```python
from build123d import *

# Parameters (mm, degrees)
HUB_BLOCK_SKETCH_R   = 32.5
HUB_BLOCK_SKETCH_R_2 = 26
HUB_BLOCK_DEPTH      = 35
ARM_PROFILE_SKETCH_R = 6.5
ARM_BODY_DEPTH       = 42


with BuildPart() as part:
    # Hub Block Sketch → Hub Block (new, symmetric)
    with BuildSketch(Plane.XY):
        Circle(HUB_BLOCK_SKETCH_R)
        Circle(HUB_BLOCK_SKETCH_R_2, mode=Mode.SUBTRACT)
    extrude(amount=HUB_BLOCK_DEPTH, both=True)

    # Arm Profile Sketch → Arm Body (add)
    with BuildSketch(Plane(origin=(0, 0, -21), x_dir=(-1, 0, 0), z_dir=(0, 0, -1))):
        with BuildLine():
            ThreePointArc((89.262059242, -14), (51.834907578, -24.492209287), (25.315908922, -52.910880046))
            ThreePointArc((25.315908922, -52.910880046), (16.763184773, -57.879874978), (7.189691393, -55.392260556))
            ThreePointArc((7.189691393, -55.392260556), (-14.44681941, -44.272249892), (-38.551485077, -40.992260556))
            ThreePointArc((-38.551485077, -40.992260556), (-49.467382276, -35.70933903), (-51.274422727, -23.717647059))
            ThreePointArc((-51.274422727, -23.717647059), (-47.255840909, 0), (-51.274422727, 23.717647059))
            ThreePointArc((-51.274422727, 23.717647059), (-49.467382276, 35.70933903), (-38.551485077, 40.992260556))
            ThreePointArc((-38.551485077, 40.992260556), (-14.44681941, 44.272249892), (7.189691393, 55.392260556))
            ThreePointArc((7.189691393, 55.392260556), (16.763184773, 57.879874978), (25.315908922, 52.910880046))
            ThreePointArc((25.315908922, 52.910880046), (51.834907578, 24.492209287), (89.262059242, 14))
            Line((89.262059242, 14), (239.5, 14))
            ThreePointArc((239.5, 14), (232.5, 0), (239.5, -14))
            Line((239.5, -14), (89.262059242, -14))
        make_face()
        with Locations((15, -45)):
            Circle(ARM_PROFILE_SKETCH_R, mode=Mode.SUBTRACT)
        with Locations((15, 45)):
            Circle(ARM_PROFILE_SKETCH_R, mode=Mode.SUBTRACT)
        with Locations((-39, -28)):
            Circle(ARM_PROFILE_SKETCH_R, mode=Mode.SUBTRACT)
        with Locations((-39, 28)):
            Circle(ARM_PROFILE_SKETCH_R, mode=Mode.SUBTRACT)
        with BuildLine():
            ThreePointArc((220, -7), (227, 0), (220, 7))
            Line((220, 7), (70, 7))
            ThreePointArc((70, 7), (63, 0), (70, -7))
            Line((70, -7), (220, -7))
        make_face(mode=Mode.SUBTRACT)
    extrude(amount=-ARM_BODY_DEPTH)


solid = part.part
```
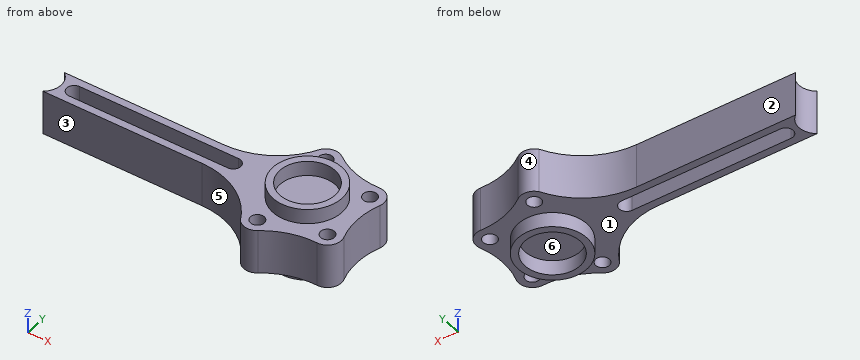
Part model, mm, in its own coordinate system. Face numbers are marked on the shaded views. A direction names the side the tool comes from. Give positions to 0.01 mm unless a question says otherwise; leave off trailing zeros. Loops run counter-clockwise (first coordinate to the right, second up) from the corner with the lowest first, then second, coordinate; pieces in that order, holes last. Notation, with made-up numbers: M 64.5,0.25 L 89.5,0.25 A18 ccw 89.5,4.25 Z; hole C 59,67.5 d5. An arc over 180 degrees is marked long. Return JSON: item names as keys, results as strings.
1) Saw through at C-C, the plane z = 15. List the corners of the cut face in (x, y).
Calculated:
{"outline": "M -239.5,-14 L -89.26,-14 A72 cw -25.32,-52.91 A13 ccw -7.19,-55.39 A72 cw 38.55,-40.99 A13 ccw 51.27,-23.72 A72 cw 51.27,23.72 A13 ccw 38.55,40.99 A72 cw -7.19,55.39 A13 ccw -25.32,52.91 A72 cw -89.26,14 L -239.5,14 A17.5 cw Z; hole M -220,-7 L -70,-7 A7 ccw -70,7 L -220,7 A7 ccw Z; hole C -15,-45 d13; hole C -15,45 d13; hole C 39,-28 d13; hole C 39,28 d13"}
2) Saw through at B-B, the plane y = 0. List the corners of the cut face in (x, z).
Calculated:
{"outline": "M -232.5,-21 L -227,-21 L -227,21 L -232.5,21 Z; M -63,-21 L -32.5,-21 L -32.5,-35 L -26,-35 L -26,-21 L 26,-21 L 26,-35 L 32.5,-35 L 32.5,-21 L 47.26,-21 L 47.26,21 L 32.5,21 L 32.5,35 L 26,35 L 26,21 L -26,21 L -26,35 L -32.5,35 L -32.5,21 L -63,21 Z"}
3) Drill centre lines: line 1 (Y direction, x = 39, z = 2); line 2 (Y direction, x = -15, z = -8); line 3 (Y direction, x = -180.5, z = 9.5). Where is each one in solid material? Low to high.
Calculated:
{"line 1": "y = -41 to -34.5, -21.5 to 21.5, 34.5 to 41", "line 2": "y = -58 to -51.5, -38.5 to 38.5, 51.5 to 58", "line 3": "y = -14 to -7, 7 to 14"}
4) Saw through at D-D, the plane x = 12.5. List the corners of the cut face in (y, z), then the cut area to 3 significant figures.
Calculated:
{"outline": "M -44.92,-21 L -30,-21 L -30,-35 L -22.8,-35 L -22.8,-21 L 22.8,-21 L 22.8,-35 L 30,-35 L 30,-21 L 44.92,-21 L 44.92,21 L 30,21 L 30,35 L 22.8,35 L 22.8,21 L -22.8,21 L -22.8,35 L -30,35 L -30,21 L -44.92,21 Z", "area": "4,180 mm2"}
5) Saw through at A-A, the plane x = -183. List the corners of the cut face in (y, z).
Calculated:
{"outline": "M -14,-21 L -7,-21 L -7,21 L -14,21 Z; M 7,-21 L 14,-21 L 14,21 L 7,21 Z"}
6) Pull direction Y, two halves, no side cores. Call the marked faces 4, 5 and 6: released by +Y, released by -Y, zero draft, split by the parting line, or undercut.
Calculated:
{"face 4": "released by +Y", "face 5": "released by -Y", "face 6": "undercut"}
7) 3-axis set-ups, long thin cutter, end or side, ignore diameter. For the marked faces 1, 2 and 3: which of +Z, -Z, +X, -X, +Y, -Y reach the whole face in a straight line?
Calculated:
{"face 1": "-Z", "face 2": "+Z, -Z, -X, +Y", "face 3": "+Z, -Z, -X, -Y"}
8) Flat gauge pins, fed straight in: pin 1 Ø10 at (x, z) = (-163, 14.5) entering from -Y; pin 2 Ø8 at (x, z) = (3, -18) entering from +Y; pin 3 Ø15.5 at (x, y) = (-11, 5) entering from +Z; pin 4 Ø8 at (x, y) = (39, -28) entering from -Z (3 decimals). Where does each tip first touch, or does it go through?
Calculated:
{"pin 1": "stops at y = -14", "pin 2": "stops at y = 51.22", "pin 3": "stops at z = 21", "pin 4": "passes through"}
